Input: part model. Units: mm. Frame: model coordinates. A direction names the side the tool comes from. Coordinates: 2 decimals unless noted, no trailing zeros. Loops run counter-clockwise (first coordinate to the right, second up) from the corner with the lowest first, then second, coordinate; pieces in that order, holes last. Notation, with made-up numbers: (5.5, -16.5) -> (20.5, -16.5) arc R26 ccw to (20.5, 10.5) -> close; hole circle Ø7 at (56.5, 74). An arc over 180 degrees is marked (long way). Answer as a JSON object with one key per item and string values.
from build123d import *

# Parameters (mm, degrees)
SKETCH_1_R      = 3
EXTRUDE_1_DEPTH = 14
SKETCH_2_R      = 2.5
EXTRUDE_2_DEPTH = 24.5
SKETCH_3_W      = 1.981719741
SKETCH_3_H      = 0.7


with BuildPart() as part:
    # 草图1 → 凸台-拉伸1 (new body)
    with BuildSketch(Plane.XY):
        Circle(SKETCH_1_R)
    extrude(amount=EXTRUDE_1_DEPTH)

    # 草图2 → 凸台-拉伸2 (add)
    with BuildSketch(Plane(origin=(0, 0, 0), x_dir=(-1, 0, 0), z_dir=(0, 0, -1))):
        with Locations(Location((0, 0, 0), (0, 0, 180))):
            Circle(SKETCH_2_R)
    extrude(amount=EXTRUDE_2_DEPTH)

    # 草图3 → 切除-旋转1 (revolve, cut)
    with BuildSketch(Plane(origin=(0, 0, 0), x_dir=(1, 0, 0), z_dir=(0, 1, 0))):
        with Locations((2.990859871, 10.35)):
            Rectangle(SKETCH_3_W, SKETCH_3_H)
    revolve(axis=Axis((0, 0, -21.474636763), (0, 0, 1)), mode=Mode.SUBTRACT)


solid = part.part
1. Access query for faces 1 (the face through (-2.5, -0.1, -17.5)), 2 (the face through (-0.26, 1.983, -10.355)), 3 (the face through (0, 0, -24.5)). Directions: +Z, -Z, +X, -X, +Y, -Y. A direction counts if a zero-diameter tool reaches every point of the face in a straight line with its end or side. Return the directions, or none.
Reply:
{"face 1": "-Z", "face 2": "none", "face 3": "-Z, +X, -X, +Y, -Y"}
2. Section query D-D (z = 2). Return loops of the section in (x, y).
Reply:
{"outline": "circle Ø6 at (0, 0)"}
3. Section query A-A (x = 0). Return loops of the section in (y, z).
Reply:
{"outline": "(-3, 0) -> (-2.5, 0) -> (-2.5, -10) -> (-2, -10) -> (-2, -10.7) -> (-2.5, -10.7) -> (-2.5, -24.5) -> (2.5, -24.5) -> (2.5, -10.7) -> (2, -10.7) -> (2, -10) -> (2.5, -10) -> (2.5, 0) -> (3, 0) -> (3, 14) -> (-3, 14) -> close"}
4. Section query B-B (y = -0.75). Return loops of the section in (x, z).
Reply:
{"outline": "(-2.9, 0) -> (-2.38, 0) -> (-2.38, -10) -> (-1.85, -10) -> (-1.85, -10.7) -> (-2.38, -10.7) -> (-2.38, -24.5) -> (2.38, -24.5) -> (2.38, -10.7) -> (1.85, -10.7) -> (1.85, -10) -> (2.38, -10) -> (2.38, 0) -> (2.9, 0) -> (2.9, 14) -> (-2.9, 14) -> close"}
5. Section query C-C (z = -18.5). Return loops of the section in (x, y).
Reply:
{"outline": "circle Ø5 at (0, 0)"}
6. Mould query, pull axis Z, two halves, no side actions, for faces 4 (the face through (-2.5, -0.1, -4.9)), 5 (the face through (1, 2, -10)), 6 (the face through (0, 0, 14)). Classes: pulls with the +Z half, pulls with the -Z half, needs draft (parallel to the pull), parting line crosses it, or undercut.
Reply:
{"face 4": "needs draft", "face 5": "undercut", "face 6": "pulls with the +Z half"}
7. Line query: line 1 along Z through (x, y) = (-0.2, -2.45); line 2 along Z through (x, y) = (2.75, 0.4); line 3 along Y through (x, z) = (1.1, -6.5) (3 decimals). Output: solid intervals per line, ascending.
Reply:
{"line 1": "z = -24.5 to -10.7, -10 to 14", "line 2": "z = 0 to 14", "line 3": "y = -2.245 to 2.245"}
8. Pin query (flat end, axial travel): P1, Ø3, axis at x = -2, z = -11, coming from the -Y side; P2, Ø2, axis at y = -2, z = 8, coming from the +X side; P3, Ø1, axis at x = -2, z = -17.5, coming from the -Y side. Return the tip coordinate at first contact, or that it passes through.
Reply:
{"P1": "stops at y = -2.45", "P2": "stops at x = 2.83", "P3": "stops at y = -2"}
